Source: CAD feature listing. Evaluate the final solid. Frame: model axes, mm. A direction names the side the tool comes from. Give positions to 0.01 mm unless a question says otherwise; leave off trailing zeros. Order: outer loops, then holes, each group sorted by start corner. A loop starts at its lowest first (then second) coordinate and runs counter-clockwise, first axis right, second up. Notation, with made-up numbers: (12.25, -38.75) - (26.25, -38.75) arc R32 cw to (26.25, -5.75) - close; hole circle Ø10 at (81, 85.25). An arc over 180 degrees is marked (long way). Write each question's results on one line, items separated by ' | '. Start each with the question number.
Item 1: Mould query, pull axis Y, two halves, no side actions, for faces 4 (the cylindrical face through (40, -20, 11)), 5 (the cylindrical face through (32.17, 12.85, 11.34)), 6 (the cylindrical face through (10.564, -40.14, 9.193)). Classes: released by +Y, released by -Y, zero draft, split by the parting line, or undercut.
Item 2: Set-up query: faces 1 (the flat face through (110, -30, 11)), 2 (the flat face through (40, -65, 11)), 3 (the cylindrical face through (57.63, -32.65, 25.46)). Return all of +Z, -Z, +X, -X, +Y, -Y with unobstructed straight access to the full face (end or side cutting, diameter ignored); none if empty.
Item 3: Contact query for flat-ended pins moving along their axis: pin 1 Ø5 at (x, y) = (46, -7) entering from +Z; pin 2 Ø7 at (x, z) = (18.5, 14) entering from +Y; pin 3 Ø16 at (x, z) = (15, 11.5) entering from -Y. Output: stop coordinate, or through.
Item 4: Section A-A on x = 7.5. Output: boundary loops of the cut face in (y, z), and give its area (3 significant figures).
Item 5: Line query: line 1 along Y through (x, z) = (65, 24.95); line 2 along Y through (x, z) = (65, 17.5); line 3 along X through (y, z) = (-40.5, 18.5). Output: solid intervals per line, ascending.
Item 6: Section C-C on z = 19.75. State how many separate pieces and enclosed holes the cut face has, and give its area (3 significant figures).
Item 7: Section B-B on y = -20. Output: boundary loops of the cut face in (x, z), and give its area (3 significant figures).
```python
from build123d import *

# Parameters (mm, degrees)
BRACKET_PROFILE_SKETCH_R = 6
BRACKET_BASE_23MM_DEPTH  = 23
BOSS_PAD_SKETCH_R        = 10
BOSS_PAD_SKETCH_R_2      = 8
BOSS_PAD_5MM_DEPTH       = 5
HOLE_10_SKETCH_R         = 5
HOLE_10_DEPTH            = 156.190205877
PROFILE_CUT_SKETCH_R     = 8
PROFILE_CUT_DEPTH        = 150.428912865


with BuildPart() as part:
    # Bracket Profile Sketch → Bracket Base 23mm (new body)
    with BuildSketch(Plane.XY):
        with BuildLine():
            Line((65, -70), (40, -70))
            Line((40, -70), (40, -60))
            ThreePointArc((40, -60), (37.071067812, -52.928932188), (30, -50))
            Line((30, -50), (0, -50))
            ThreePointArc((0, -50), (-10, -40), (0, -30))
            Line((0, -30), (30, -30))
            ThreePointArc((30, -30), (40, -20), (30, -10))
            Line((30, -10), (0, -10))
            ThreePointArc((0, -10), (-10, 0), (0, 10))
            Line((0, 10), (25.18, 10))
            ThreePointArc((25.18, 10), (32.251067812, 12.928932188), (35.18, 20))
            Line((35.18, 20), (35.18, 30))
            Line((35.18, 30), (65, 30))
            ThreePointArc((65, 30), (79.174121887, 24.110280263), (85, 9.910000911))
            Line((85, 9.910000911), (84.955100778, -0.067604024))
            ThreePointArc((84.955100778, -0.067604024), (87.883932045, -7.183671708), (95, -10.112502316))
            Line((95, -10.112502316), (120, -10))
            ThreePointArc((120, -10), (130, -20), (120, -30))
            Line((120, -30), (99.82, -30))
            ThreePointArc((99.82, -30), (92.748932188, -32.928932188), (89.82, -40))
            Line((89.82, -40), (89.82, -50))
            ThreePointArc((89.82, -50), (83.962135624, -64.142135624), (69.82, -70))
            Line((69.82, -70), (65, -70))
        make_face()
        Circle(BRACKET_PROFILE_SKETCH_R, mode=Mode.SUBTRACT)
        with Locations((0, -40)):
            Circle(BRACKET_PROFILE_SKETCH_R, mode=Mode.SUBTRACT)
        with BuildLine():
            Line((120, -26), (65, -26))
            ThreePointArc((65, -26), (59, -20), (65, -14))
            Line((65, -14), (120, -14))
            ThreePointArc((120, -14), (126, -20), (120, -26))
        make_face(mode=Mode.SUBTRACT)
    extrude(amount=BRACKET_BASE_23MM_DEPTH)

    # Boss Pad Sketch → Boss Pad 5mm (add)
    # profile 1 of 2: a face of its own
    with BuildSketch(Plane.XY.offset(23)):
        with Locations((65, 10)):
            Circle(BOSS_PAD_SKETCH_R)
        with Locations((65, 10)):
            Circle(BOSS_PAD_SKETCH_R_2, mode=Mode.SUBTRACT)
    # profile 2 of 2: a face of its own
    with BuildSketch(Plane.XY.offset(23)):
        with Locations((65, -39.411185403)):
            Circle(BOSS_PAD_SKETCH_R)
        with Locations((65, -39.411185403)):
            Circle(BOSS_PAD_SKETCH_R_2, mode=Mode.SUBTRACT)
    extrude(amount=BOSS_PAD_5MM_DEPTH)

    # Hole Ø10 Sketch → Hole Ø10 (cut, through all)
    with BuildSketch(Plane.XZ.offset(50)):
        with Locations(Location((15, 11.5, 0), (0, 0, 270))):
            Circle(HOLE_10_SKETCH_R)
    extrude(amount=-HOLE_10_DEPTH, mode=Mode.SUBTRACT)

    # Profile Cut Sketch → Profile Cut (cut, through all)
    with BuildSketch(Plane.XY.offset(23)):
        with Locations((65, 10)):
            Circle(PROFILE_CUT_SKETCH_R)
        with Locations((65, -39.411185403)):
            Circle(PROFILE_CUT_SKETCH_R)
    extrude(amount=-PROFILE_CUT_DEPTH, mode=Mode.SUBTRACT)


solid = part.part
```
Evaluation:
1) face 4: undercut | face 5: released by +Y | face 6: zero draft
2) face 1: +Z, -Z, +X, -Y | face 2: +Z, -Z, -X, -Y | face 3: +Z
3) pin 1: stops at z = 23 | pin 2: stops at y = 10 | pin 3: stops at y = -50
4) outline: (-50, 0) - (-30, 0) - (-30, 23) - (-50, 23) - close; (-10, 0) - (10, 0) - (10, 23) - (-10, 23) - close | area: 920 mm^2
5) line 1: y = -49.41 to -47.41, -31.41 to -29.41, 0 to 2, 18 to 20 | line 2: y = -70 to -47.41, -31.41 to -26, -14 to 2, 18 to 30 | line 3: x = -9.99 to -5.98, 5.98 to 57.07, 72.93 to 89.82
6) separate pieces: 1 | enclosed holes: 5 | area: 6,110 mm^2
7) outline: (40, 0) - (59, 0) - (59, 23) - (40, 23) - close; (126, 0) - (130, 0) - (130, 23) - (126, 23) - close | area: 529 mm^2
